Can you work these out from the model? Positions are in its coordinate system, mm. Round coordinates to 2 decimals unless told otherwise and drop trailing zeros. Order: outer loops, then holes, each group sorted by start corner. A loop starts at its lowest first (then second) coordinate and runs counter-clockwise, first axis right, second up. Notation, with made-up numbers: (45, -21.75) -> (58, -21.75) arc R14 cw to (58, -16.75) -> close; hole circle Ø11 at (-13.5, 71). An arc over 180 degrees is marked (long way). Use a Markdown table: item, result. Add a question column.
Q1. I need wall thicknesses on line 1 along X through (y, z) = (-260, 6.75); line 2 along Y through (x, z) = (34, 7.5); line 3 along Y through (x, z) = (-33.5, 5.5). Which ranges of each line are inside material? Lowest first, please. Write a range as [from, to].
Q2. If we section it at C-C on y = -190: List the corners of the cut face in (x, z) for me.
Q3. If we section it at A-A on y = 169.5: List the corners of the cut face in (x, z) for me, plus the area to 3 significant figures.
Q4. If we section it at B-B on z = 7.25: List the corners of the cut face in (x, y) for me.
Q5. I'm going to push a flat-ended pin straight in: pin 1 Ø6 at (x, y) = (-35, -190) entering from -Z. Where does the tip first touch, or does it pass through?
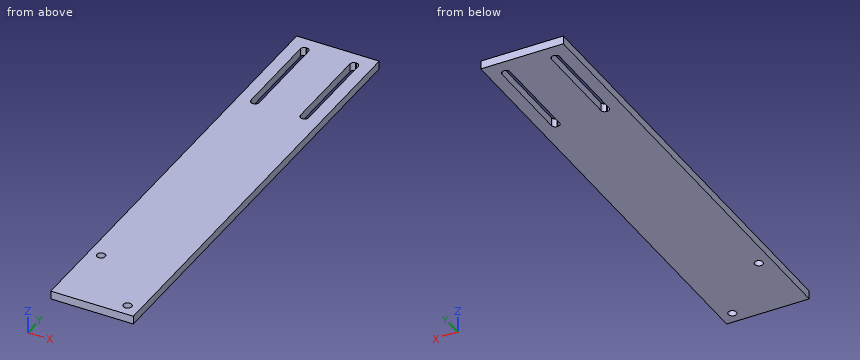
```python
from build123d import *

# Parameters (mm, degrees)
SKETCH1_W           = 100
SKETCH1_H           = 550
BOSS_EXTRUDE1_DEPTH = 10
SKETCH2_R           = 5
CUT_EXTRUDE1_DEPTH  = 10
CUT_EXTRUDE2_DEPTH  = 10


with BuildPart() as part:
    # Sketch1 → Boss-Extrude1 (new body)
    with BuildSketch(Plane.XY):
        Rectangle(SKETCH1_W, SKETCH1_H)
    extrude(amount=BOSS_EXTRUDE1_DEPTH)

    # Sketch2 → Cut-Extrude1 (cut)
    with BuildSketch(Plane.XY.offset(10)):
        with Locations((-35, -190)):
            Circle(SKETCH2_R)
        with Locations((35, -260)):
            Circle(SKETCH2_R)
    extrude(amount=-CUT_EXTRUDE1_DEPTH, mode=Mode.SUBTRACT)

    # Sketch3 → Cut-Extrude2 (cut)
    with BuildSketch(Plane.XY.offset(10)):
        with BuildLine():
            Line((-29.5, 140.099701054), (-30.5, 140.099701054))
            ThreePointArc((-30.5, 140.099701054), (-33.681980515, 141.417720539), (-35, 144.599701054))
            Line((-35, 144.599701054), (-35, 255.599701054))
            ThreePointArc((-35, 255.599701054), (-33.681980515, 258.78168157), (-30.5, 260.099701054))
            Line((-30.5, 260.099701054), (-29.5, 260.099701054))
            ThreePointArc((-29.5, 260.099701054), (-26.318019485, 258.78168157), (-25, 255.599701054))
            Line((-25, 255.599701054), (-25, 144.599701054))
            ThreePointArc((-25, 144.599701054), (-26.318019485, 141.417720539), (-29.5, 140.099701054))
        make_face()
        with BuildLine():
            Line((30.5, 140.099701054), (29.5, 140.099701054))
            ThreePointArc((29.5, 140.099701054), (26.318019485, 141.417720539), (25, 144.599701054))
            Line((25, 144.599701054), (25, 255.599701054))
            ThreePointArc((25, 255.599701054), (26.318019485, 258.78168157), (29.5, 260.099701054))
            Line((29.5, 260.099701054), (30.5, 260.099701054))
            ThreePointArc((30.5, 260.099701054), (33.681980515, 258.78168157), (35, 255.599701054))
            Line((35, 255.599701054), (35, 144.599701054))
            ThreePointArc((35, 144.599701054), (33.681980515, 141.417720539), (30.5, 140.099701054))
        make_face()
    extrude(amount=-CUT_EXTRUDE2_DEPTH, mode=Mode.SUBTRACT)


solid = part.part
```
Answer below:
| question | item | result |
|---|---|---|
| 1 | line 1 | [-50, 30], [40, 50] |
| 1 | line 2 | [-275, -264.9], [-255.1, 141.77], [258.43, 275] |
| 1 | line 3 | [-275, -194.77], [-185.23, 141.25], [258.95, 275] |
| 2 | outline | (-50, 0) -> (-40, 0) -> (-40, 10) -> (-50, 10) -> close; (-30, 0) -> (50, 0) -> (50, 10) -> (-30, 10) -> close |
| 3 | outline | (-50, 0) -> (-35, 0) -> (-35, 10) -> (-50, 10) -> close; (-25, 0) -> (25, 0) -> (25, 10) -> (-25, 10) -> close; (35, 0) -> (50, 0) -> (50, 10) -> (35, 10) -> close |
| 3 | area | 800 mm² |
| 4 | outline | (-50, -275) -> (50, -275) -> (50, 275) -> (-50, 275) -> close; hole circle Ø10 at (-35, -190); hole (-35, 144.6) arc R4.5 ccw to (-30.5, 140.1) -> (-29.5, 140.1) arc R4.5 ccw to (-25, 144.6) -> (-25, 255.6) arc R4.5 ccw to (-29.5, 260.1) -> (-30.5, 260.1) arc R4.5 ccw to (-35, 255.6) -> close; hole (25, 144.6) arc R4.5 ccw to (29.5, 140.1) -> (30.5, 140.1) arc R4.5 ccw to (35, 144.6) -> (35, 255.6) arc R4.5 ccw to (30.5, 260.1) -> (29.5, 260.1) arc R4.5 ccw to (25, 255.6) -> close; hole circle Ø10 at (35, -260) |
| 5 | pin 1 | through |
